Input: part model. Units: mm. Frame: model coordinates. Face numbers are marked on the shaded views. A direction names the side the tool comes from. Give positions to 0.01 mm unless a question says otherwise; leave off trailing zeros. Loops run counter-clockwise (first coordinate to the right, second up) from the corner with the lowest first, then second, coordinate; pieces in that order, holes last. Notation, with made-up numbers: (-32.5, 83.5) -> (-14.5, 83.5) arc R20 cw to (-14.5, 99.5) -> close; hole circle Ø2 at (-1.75, 70.25). An arc over 180 degrees is marked (long way). Answer in a Markdown table with one row per item. Add a question column.
```python
from build123d import *

# Parameters (mm, degrees)
SKETCH1_W           = 400
SKETCH1_H           = 450
BOSS_EXTRUDE1_DEPTH = 600
SKETCH2_W           = 440
SKETCH2_H           = 490
BOSS_EXTRUDE2_DEPTH = 20
SKETCH3_W           = 400
SKETCH3_H           = 5
CUT_EXTRUDE1_DEPTH  = 5
SKETCH4_W           = 400
SKETCH4_H           = 5
CUT_EXTRUDE2_DEPTH  = 5
SKETCH5_W           = 100
SKETCH5_H           = 10
BOSS_EXTRUDE3_DEPTH = 20
SKETCH6_W           = 100
SKETCH6_H           = 10
BOSS_EXTRUDE4_DEPTH = 20
SKETCH7_W           = 100
SKETCH7_H           = 10
BOSS_EXTRUDE5_DEPTH = 20
SKETCH8_W           = 90
SKETCH8_H           = 14.666116079
CUT_EXTRUDE3_DEPTH  = 500


with BuildPart() as part:
    # Sketch1 → Boss-Extrude1 (new body)
    with BuildSketch(Plane.XY):
        with Locations((200, 225)):
            Rectangle(SKETCH1_W, SKETCH1_H)
    extrude(amount=BOSS_EXTRUDE1_DEPTH)

    # Sketch2 → Boss-Extrude2 (add)
    with BuildSketch(Plane.XY.offset(600)):
        with Locations((200, 225)):
            Rectangle(SKETCH2_W, SKETCH2_H)
    extrude(amount=-BOSS_EXTRUDE2_DEPTH)

    # Sketch3 → Cut-Extrude1 (cut)
    with BuildSketch(Plane.XZ):
        with Locations((200, 437.5)):
            Rectangle(SKETCH3_W, SKETCH3_H)
    extrude(amount=-CUT_EXTRUDE1_DEPTH, mode=Mode.SUBTRACT)

    # Sketch4 → Cut-Extrude2 (cut)
    with BuildSketch(Plane.XZ):
        with Locations((200, 282.5)):
            Rectangle(SKETCH4_W, SKETCH4_H)
    extrude(amount=-CUT_EXTRUDE2_DEPTH, mode=Mode.SUBTRACT)

    # Sketch5 → Boss-Extrude3 (add)
    with BuildSketch(Plane.XZ):
        with Locations((200, 510)):
            Rectangle(SKETCH5_W, SKETCH5_H)
    extrude(amount=BOSS_EXTRUDE3_DEPTH)

    # Sketch6 → Boss-Extrude4 (add)
    with BuildSketch(Plane.XZ):
        with Locations((200, 360)):
            Rectangle(SKETCH6_W, SKETCH6_H)
    extrude(amount=BOSS_EXTRUDE4_DEPTH)

    # Sketch7 → Boss-Extrude5 (add)
    with BuildSketch(Plane.XZ):
        with Locations((200, 155)):
            Rectangle(SKETCH7_W, SKETCH7_H)
    extrude(amount=BOSS_EXTRUDE5_DEPTH)

    # Sketch8 → Cut-Extrude3 (cut)
    with BuildSketch(Plane.XY.offset(515)):
        with Locations((200, -7.666941961)):
            Rectangle(SKETCH8_W, SKETCH8_H)
    extrude(amount=-CUT_EXTRUDE3_DEPTH, mode=Mode.SUBTRACT)


solid = part.part
```
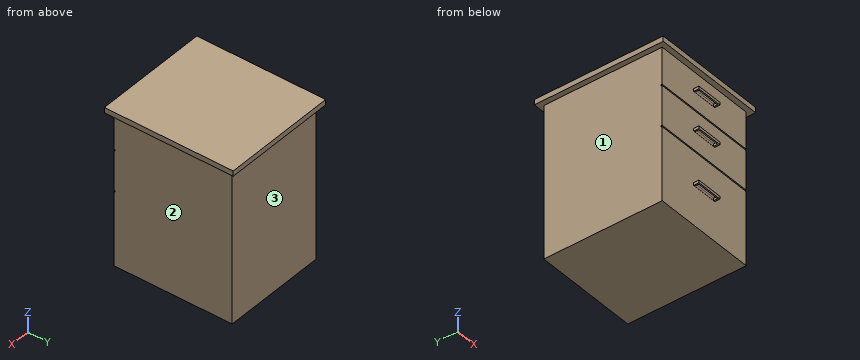
1) Section B-B on y = 287.5. Output: boundary loops of the cut face in (x, z).
2) Pin query (flat end, axial travel): pin 1 (8 mm diameter, centred on y = -6.5, z = 156, fed in from +X); pin 2 (6 mm diameter, centred on y = 147, z = 141, fed in from -X); pin 3 (8 mm diameter, centred on x = 167, z = 340, fed in from +Y). Return the tip coordinate at first contact, or that it passes through.
3) Reachability of the marked faces 1, 2 and 3 from +Z, -Z, +X, -X, +Y, -Y: full face, straight path, thin tool, end or side. Return the list, or none.
4) Section A-A on x = 54. Output: boundary loops of the cut face in (y, z), and give its area (3 significant figures).
5) Section D-D on z = 53. Output: boundary loops of the cut face in (x, y).
6) Material intervals for line 1 along X through (y, z) = (35, 234.5); line 2 along Y through (x, z) = (44, 199.5), sorted ascending.
7) Section C-C on x = 185.5. State how many separate pieces and enclosed holes the cut face has, and give its area (3 significant figures).
Working result:
| question | item | result |
|---|---|---|
| 1 | outline | (-20, 580) -> (0, 580) -> (0, 0) -> (400, 0) -> (400, 580) -> (420, 580) -> (420, 600) -> (-20, 600) -> close |
| 2 | pin 1 | stops at x = 250 |
| 2 | pin 2 | stops at x = 0 |
| 2 | pin 3 | stops at y = 450 |
| 3 | face 1 | -Z, -X, +Y, -Y |
| 3 | face 2 | -Z, +X, +Y, -Y |
| 3 | face 3 | -Z, +X, -X, +Y |
| 4 | outline | (-20, 580) -> (0, 580) -> (0, 440) -> (5, 440) -> (5, 435) -> (0, 435) -> (0, 285) -> (5, 285) -> (5, 280) -> (0, 280) -> (0, 0) -> (450, 0) -> (450, 580) -> (470, 580) -> (470, 600) -> (-20, 600) -> close |
| 4 | area | 271,000 mm2 |
| 5 | outline | (0, 0) -> (400, 0) -> (400, 450) -> (0, 450) -> close |
| 6 | line 1 | x = 0 to 400 |
| 6 | line 2 | y = 0 to 450 |
| 7 | separate pieces | 4 |
| 7 | enclosed holes | 0 |
| 7 | area | 271,000 mm2 |
